Geometry check sheet. Reference: the model listing, model coordinates, mm. Face numbers are marked on the shaded views. A direction names the side the tool comes from. Coordinates: 2 decimals unless noted, no trailing zeros. Write each loop counter-clockwise with the first axis right and the second up, starting at its lowest first coordinate (ties: lowest second). Pieces come first, ordered by that corner, then holes. Notation, with made-up numbers: M -37.5,80.25 L -12.5,80.25 A29 cw -12.5,101.25 Z; hole C 3.5,10 d9. An arc over 180 degrees is marked long. Answer as a JSON object with one key per item and string values. Group by question number.
```python
from build123d import *

# Parameters (mm, degrees)
SKETCH1_W           = 50
SKETCH1_H           = 50
BOSS_EXTRUDE2_DEPTH = 150
SKETCH2_W           = 30
SKETCH2_H           = 50
CUT_EXTRUDE1_DEPTH  = 35
SKETCH4_R           = 16
CUT_EXTRUDE2_DEPTH  = 10
SKETCH5_R           = 4
CUT_EXTRUDE3_DEPTH  = 10


with BuildPart() as part:
    # Sketch1 → Boss-Extrude2 (new body)
    with BuildSketch(Plane(origin=(0, 0, 0), x_dir=(1, 0, 0), z_dir=(0, 1, 0))):
        Rectangle(SKETCH1_W, SKETCH1_H)
    extrude(amount=BOSS_EXTRUDE2_DEPTH)

    # Sketch2 → Cut-Extrude1 (cut)
    with BuildSketch(Plane.XZ):
        Rectangle(SKETCH2_W, SKETCH2_H)
    extrude(amount=-CUT_EXTRUDE1_DEPTH, mode=Mode.SUBTRACT)

    # Sketch4 → Cut-Extrude2 (cut)
    with BuildSketch(Plane(origin=(0, 150, 0), x_dir=(1, 0, 0), z_dir=(0, 1, 0))):
        with Locations(Location((0, 0, 0), (0, 0, 270))):
            Circle(SKETCH4_R)
    extrude(amount=-CUT_EXTRUDE2_DEPTH, mode=Mode.SUBTRACT)

    # Sketch5 → Cut-Extrude3 (cut)
    with BuildSketch(Plane(origin=(25, 0, 0), x_dir=(0, 0, -1), z_dir=(1, 0, 0))):
        with Locations((-16, 130)):
            Circle(SKETCH5_R)
        with Locations((16, 130)):
            Circle(SKETCH5_R)
        with Locations((-16, 90)):
            Circle(SKETCH5_R)
        with Locations((-16, 50)):
            Circle(SKETCH5_R)
        with Locations((16, 50)):
            Circle(SKETCH5_R)
        with Locations(Location((16, 90, 0), (0, 0, 180))):
            Circle(SKETCH5_R)
    cut_extrude3 = extrude(amount=-CUT_EXTRUDE3_DEPTH, mode=Mode.SUBTRACT)

    # Mirror1: Cut-Extrude3 across plane
    add(cut_extrude3.mirror(Plane(origin=(0, 0, 0), x_dir=(0, 0, 1), z_dir=(1, 0, 0))), mode=Mode.SUBTRACT)


solid = part.part
```
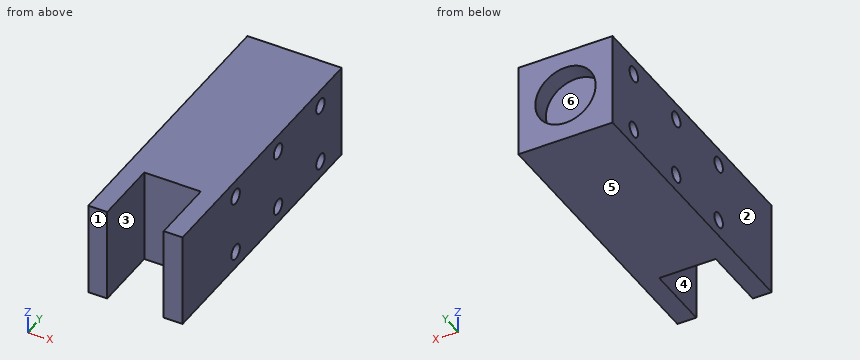
1) Section check D-D (z = 10). Record the cut outline in (x, y).
2) Set-up check for the marked faces 4, 5 and 6: record each of +Z, -Z, +X, -X, +Y, -Y from which the full face is reachable in a straight line by a thin tool's end or side.
3) Section check C-C (y = 130). Record the cut outline in (x, z), then the cut area to 3 significant figures.
4) Draft check along X on the marked faces 1, 2 and 3. Enter one of: +X half, -X half, draft (parallel to the pull), parting line (faces both ways), or undercut.
5) Section check B-B (x = 22.5). Record the cut outline in (y, z), then the cut area to 3 significant figures.
6) Go/stop test with flat-tipped pins: pin 1 Ø7 at (y, z) = (130, -16) entering from -X; pin 2 Ø9.5 at (x, z) = (-1.5, -4) entering from +Y; pin 3 Ø4 at (y, z) = (130, 14.5) entering from +X. Record where each tip stops, or that it passes through.
7) Material ranges on probe 1 along Y at (x, z) = (21.75, -16); probe 2 along X at (y, z) = (33, -0.5); probe 3 along Z at (x, y) = (-21, 46.5), recorded low to high. Write a range as [from, to].
8) Section check A-A (y = 25). Record the cut outline in (x, z).
Entries:
{
 "1": {"outline": "M -25,0 L -15,0 L -15,35 L 15,35 L 15,0 L 25,0 L 25,150 L 12.49,150 L 12.49,140 L -12.49,140 L -12.49,150 L -25,150 Z"},
 "2": {"face 4": "+Z, -Z, -Y", "face 5": "-Z, +X, -X, +Y, -Y", "face 6": "+Y"},
 "3": {"outline": "M -25,-25 L 25,-25 L 25,-20 L 15,-20 L 15,-12 L 25,-12 L 25,12 L 15,12 L 15,20 L 25,20 L 25,25 L -25,25 L -25,20 L -15,20 L -15,12 L -25,12 L -25,-12 L -15,-12 L -15,-20 L -25,-20 Z", "area": "2,180 mm^2"},
 "4": {"face 1": "draft", "face 2": "-X half", "face 3": "undercut"},
 "5": {"outline": "M 0,-25 L 150,-25 L 150,25 L 0,25 Z; hole C 50,-16 d8; hole C 50,16 d8; hole C 90,-16 d8; hole C 90,16 d8; hole C 130,-16 d8; hole C 130,16 d8", "area": "7,200 mm^2"},
 "6": {"pin 1": "x = -15", "pin 2": "y = 140", "pin 3": "x = 15"},
 "7": {"probe 1": "[0, 46], [54, 86], [94, 126], [134, 150]", "probe 2": "[-25, -15], [15, 25]", "probe 3": "[-25, -17.94], [-14.06, 14.06], [17.94, 25]"},
 "8": {"outline": "M -25,-25 L -15,-25 L -15,25 L -25,25 Z; M 15,-25 L 25,-25 L 25,25 L 15,25 Z"}
}
